Input: part model. Units: mm. Frame: model coordinates. Face numbers are marked on the shaded views. A direction names the side the tool comes from. Round coordinates to 2 decimals unless told otherwise and drop trailing zeros. Loops run counter-clockwise (first coordinate to the right, second up) from the corner with the lowest first, then second, coordinate; pieces in that order, holes last. Notation, with made-up numbers: (-22, 83.25) - (29, 83.25) arc R34 ccw to (29, 113.25) - close; hole circle Ø2 at (66.5, 8.25). An arc over 180 degrees is marked (long way). One line per question, with ' | ' between items. Start each with the question number.
Item 1: Section C-C, the plane y = 14. Return loops of the section in (x, z).
Item 2: Section D-D, the plane z = -75.5. Return loops of the section in (x, y).
Item 3: First-contact query: pin 1 (8 mm diameter, centred on x = 10, z = 34, fed in from +Y); pin 2 (6.5 mm diameter, centred on x = 43, z = -75.5, fed in from -Y); pin 3 (9 mm diameter, centred on y = 5.5, z = -89, fed in from +X). Flat tips, straight axial feed; report the tip coordinate or a pass-through.
Item 4: Section B-B, the plane z = 0. Return loops of the section in (x, y), plus the area to 3 significant figures.
Item 5: Draft query along X for the marked faces 1, 2 and 3. Return one class per face: pulls with the +X half, pulls with the -X half, needs draft (parallel to the pull), parting line crosses it, or undercut.
Item 6: Set-up query: the marked faces 4 and 5. Return all of +Z, -Z, +X, -X, +Y, -Y with unobstructed straight access to the full face (end or side cutting, diameter ignored); none if empty.
Item 7: Material intervals for line 1 along X through (y, z) = (5, 66); line 2 along X through (y, z) = (1, -75); line 3 along Y through (x, z) = (68.05, 0), sorted ascending.
Item 8: Section A-A, the plane x = -23. Return loops of the section in (y, z).
```python
from build123d import *

# Parameters (mm, degrees)
SKETCH1_W                = 138
SKETCH1_H                = 160
BOSS_EXTRUDE1_DEPTH      = 8
SKETCH9_W                = 30
SKETCH9_H                = 38
SKETCH9_R                = 3.4
SKETCH9_R_2              = 1.5
BOSS_EXTRUDE4_DEPTH      = 3
RIB2_REACH               = 165.976
SKETCH10_WALL_W          = 364.592232036
SKETCH10_WALL_H          = 3
MIRROR4_COPY_1_REACH     = 165.976
MIRROR4_COPY_1_SKETCH_W  = 364.592232036
MIRROR4_COPY_1_SKETCH_H  = 3
CUT_EXTRUDE2_DEPTH       = 110.822584198
CUT_EXTRUDE2_DEPTH_BACK  = 110.822584198
SKETCH11_R               = 1.5
FILLET1_R                = 5
SKETCH12_R               = 1.75
CUT_EXTRUDE3_DEPTH       = 110.822584198
CUT_EXTRUDE4_DEPTH       = 110.822584198
BOSS_EXTRUDE5_DEPTH      = 60
BOSS_EXTRUDE5_DEPTH_BACK = 60
CUT_EXTRUDE5_DEPTH       = 137.926987844
CUT_EXTRUDE5_DEPTH_BACK  = 137.926987844
SKETCH15_R               = 2
SKETCH16_R               = 1.75
CUT_EXTRUDE6_DEPTH       = 50


with BuildPart() as part:
    # Sketch1 → Boss-Extrude1 (new body)
    with BuildSketch(Plane(origin=(0, 0, 0), x_dir=(1, 0, 0), z_dir=(0, 1, 0))):
        Rectangle(SKETCH1_W, SKETCH1_H)
    extrude(amount=BOSS_EXTRUDE1_DEPTH)

    # Sketch9 → Boss-Extrude4 (add)
    with BuildSketch(Plane.ZY.offset(69)):
        with Locations((0, 19)):
            Rectangle(SKETCH9_W, SKETCH9_H)
        with Locations((0, 23)):
            Circle(SKETCH9_R, mode=Mode.SUBTRACT)
        with Locations((8.5, 23)):
            Circle(SKETCH9_R_2, mode=Mode.SUBTRACT)
        with Locations((-8.5, 23)):
            Circle(SKETCH9_R_2, mode=Mode.SUBTRACT)
    boss_extrude4 = extrude(amount=-BOSS_EXTRUDE4_DEPTH)

    # Sketch10 wall → Rib2 (add, up to next)
    with BuildSketch(Plane(origin=(-69, 23, -23.660254038), x_dir=(0, -0.866025403781, -0.500000000007), z_dir=(0, -0.500000000007, 0.866025403781)), mode=Mode.PRIVATE) as rib2_sk1:
        with Locations((0, 1.5)):
            Rectangle(SKETCH10_WALL_W, SKETCH10_WALL_H)
    rib2_tool1 = extrude(rib2_sk1.sketch, amount=RIB2_REACH, mode=Mode.PRIVATE) - part.part
    rib2 = rib2_tool1.solids().sort_by_distance((-69, 23, -23.660254038))[0]
    add(rib2)

    # Mirror3: Rib2 across plane
    add(rib2.mirror(Plane.XY))

    # Mirror4: Boss-Extrude4, Rib2 across plane
    add(boss_extrude4.mirror(Plane(origin=(0, 0, 0), x_dir=(0, 0, 1), z_dir=(1, 0, 0))))
    add(rib2.mirror(Plane(origin=(0, 0, 0), x_dir=(0, 0, 1), z_dir=(1, 0, 0))))

    # Mirror4 copy 1 sketch → Mirror4 copy 1 (add, up to next)
    with BuildSketch(Plane(origin=(69, 23, 23.660254038), x_dir=(0, -0.866025403781, 0.500000000007), z_dir=(0, -0.500000000007, -0.866025403781)), mode=Mode.PRIVATE) as mirror4_copy_1_sk1:
        with Locations((0, 1.5)):
            Rectangle(MIRROR4_COPY_1_SKETCH_W, MIRROR4_COPY_1_SKETCH_H)
    mirror4_copy_1_tool1 = extrude(mirror4_copy_1_sk1.sketch, amount=MIRROR4_COPY_1_REACH, mode=Mode.PRIVATE) - part.part
    add(mirror4_copy_1_tool1.solids().sort_by_distance((69, 23, 23.660254038))[0])

    # Sketch11 → Cut-Extrude2 (cut, two sides: drawn at the far end of the back side and taken through both)
    with BuildSketch(Plane(origin=(0, 8, 0), x_dir=(1, 0, 0), z_dir=(0, 1, 0)).offset(-CUT_EXTRUDE2_DEPTH_BACK)):
        with Locations(Location((-28.95, -24.1, 0), (0, 0, 270))):
            Circle(SKETCH11_R)
        with Locations(Location((28.95, -24.1, 0), (0, 0, 90))):
            Circle(SKETCH11_R)
        with Locations(Location((-28.95, -66, 0), (0, 0, 90))):
            Circle(SKETCH11_R)
        with Locations(Location((28.95, -66, 0), (0, 0, 270))):
            Circle(SKETCH11_R)
    extrude(amount=CUT_EXTRUDE2_DEPTH + CUT_EXTRUDE2_DEPTH_BACK, mode=Mode.SUBTRACT)

    # Fillet1
    fillet1_edges = [part.edges().sort_by_distance(p)[0] for p in [
        (69, 4, 80),
        (-69, 4, 80),
        (-69, 4, -80),
        (69, 4, -80),
    ]]
    fillet(fillet1_edges, radius=FILLET1_R)

    # Sketch12 → Cut-Extrude3 (cut, symmetric)
    with BuildSketch(Plane(origin=(0, 8, 0), x_dir=(1, 0, 0), z_dir=(0, 1, 0))):
        with Locations(Location((64.5, -55, 0), (0, 0, 270))):
            Circle(SKETCH12_R)
        with Locations(Location((64.5, -68, 0), (0, 0, 270))):
            Circle(SKETCH12_R)
    cut_extrude3 = extrude(amount=CUT_EXTRUDE3_DEPTH, both=True, mode=Mode.SUBTRACT)

    # Mirror5: Cut-Extrude3 across plane
    add(cut_extrude3.mirror(Plane(origin=(0, 0, 0), x_dir=(0, 0, 1), z_dir=(1, 0, 0))), mode=Mode.SUBTRACT)

    # Sketch13 → Cut-Extrude4 (cut, symmetric)
    with BuildSketch(Plane(origin=(0, 8, 0), x_dir=(1, 0, 0), z_dir=(0, 1, 0))):
        with BuildLine():
            Line((60, 80), (80.385419548, 90.585690096))
            Line((80.385419548, 90.585690096), (122.100847158, 60.329129947))
            Line((122.100847158, 60.329129947), (69, 36.320508076))
            ThreePointArc((69, 36.320508076), (61.687085415, 57.580663247), (60, 80))
        make_face()
    cut_extrude4 = extrude(amount=CUT_EXTRUDE4_DEPTH, both=True, mode=Mode.SUBTRACT)

    # Mirror6: Cut-Extrude4 across plane
    add(cut_extrude4.mirror(Plane(origin=(0, 0, 0), x_dir=(0, 0, 1), z_dir=(1, 0, 0))), mode=Mode.SUBTRACT)

    # Sketch14 → Boss-Extrude5 (add, two sides: drawn at the far end of the back side and taken through both)
    with BuildSketch(Plane(origin=(0, 0, 0), x_dir=(0, 0, -1), z_dir=(1, 0, 0)).offset(-BOSS_EXTRUDE5_DEPTH_BACK)):
        Polygon((80, 0), (80, 8), (112, 0), align=None)
    extrude(amount=BOSS_EXTRUDE5_DEPTH + BOSS_EXTRUDE5_DEPTH_BACK)

    # Sketch15 → Cut-Extrude5 (cut, two sides: drawn at the far end of the back side and taken through both)
    with BuildSketch(Plane.XZ.offset(-CUT_EXTRUDE5_DEPTH_BACK)):
        with Locations(Location((-45, -75.5, 0), (0, 0, 270))):
            Circle(SKETCH15_R)
        with Locations(Location((-23, -75.5, 0), (0, 0, 270))):
            Circle(SKETCH15_R)
        with Locations(Location((-1, -75.5, 0), (0, 0, 270))):
            Circle(SKETCH15_R)
        with Locations(Location((21, -75.5, 0), (0, 0, 270))):
            Circle(SKETCH15_R)
        with Locations(Location((43, -75.5, 0), (0, 0, 270))):
            Circle(SKETCH15_R)
    extrude(amount=CUT_EXTRUDE5_DEPTH + CUT_EXTRUDE5_DEPTH_BACK, mode=Mode.SUBTRACT)

    # Sketch16 → Cut-Extrude6 (cut)
    with BuildSketch(Plane(origin=(0, 8, 0), x_dir=(1, 0, 0), z_dir=(0, 1, 0))):
        with Locations(Location((0, 37, 0), (0, 0, 270))):
            Circle(SKETCH16_R)
        with Locations(Location((18, 37, 0), (0, 0, 270))):
            Circle(SKETCH16_R)
        with Locations(Location((-18, 37, 0), (0, 0, 90))):
            Circle(SKETCH16_R)
    extrude(amount=-CUT_EXTRUDE6_DEPTH, mode=Mode.SUBTRACT)


solid = part.part
```
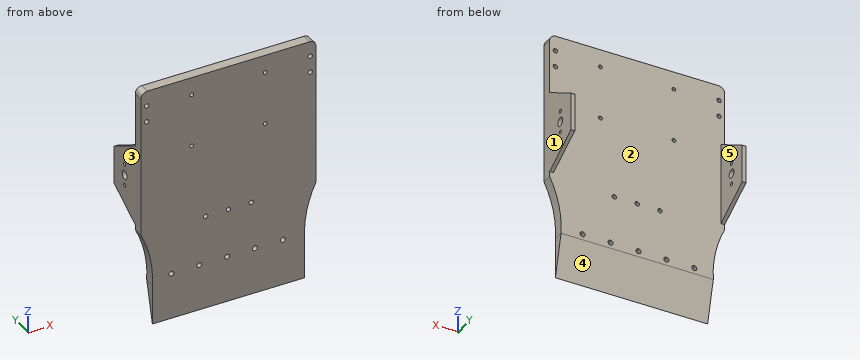
Return value:
1) outline: (-69, -28.86) - (-66, -28.86) - (-66, 28.86) - (-69, 28.86) - close; (66, -28.86) - (69, -28.86) - (69, 28.86) - (66, 28.86) - close
2) outline: (-59.88, 0) - (-47, 0) - (-47, 8) - (-59.88, 8) - close; (-43, 0) - (-25, 0) - (-25, 8) - (-43, 8) - close; (-21, 0) - (-3, 0) - (-3, 8) - (-21, 8) - close; (1, 0) - (19, 0) - (19, 8) - (1, 8) - close; (23, 0) - (41, 0) - (41, 8) - (23, 8) - close; (45, 0) - (59.88, 0) - (59.88, 8) - (45, 8) - close
3) pin 1: y = 8 | pin 2: y = 0 | pin 3: x = 60
4) outline: (-69, 0) - (69, 0) - (69, 19.6) - (66, 19.6) - (66, 8) - (-66, 8) - (-66, 19.6) - (-69, 19.6) - close; (-69, 26.4) - (-66, 26.4) - (-66, 38) - (-69, 38) - close; (66, 26.4) - (69, 26.4) - (69, 38) - (66, 38) - close | area: 1,240 mm2
5) face 1: pulls with the +X half | face 2: undercut | face 3: pulls with the -X half
6) face 4: -Z, +X, -X, +Y | face 5: +Z, -Z, +Y
7) line 1: -69 to -30.45, -27.45 to 27.45, 30.45 to 69 | line 2: -59.88 to -46.94, -43.06 to -24.94, -21.06 to -2.94, 0.94 to 19.06, 22.94 to 41.06, 44.94 to 59.88 | line 3: 0 to 19.6, 26.4 to 38
8) outline: (0, -112) - (8, -80) - (8, -77.5) - (0, -77.5) - close; (0, -73.5) - (8, -73.5) - (8, 80) - (0, 80) - close
